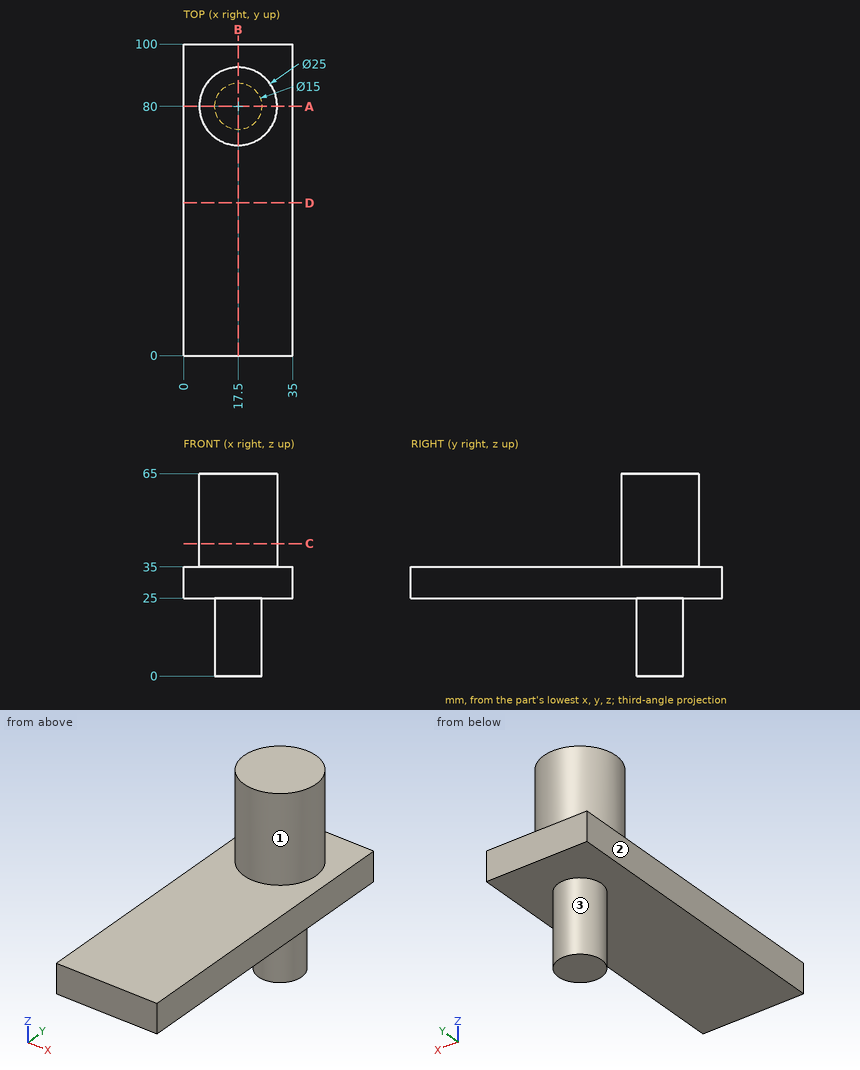
Here's the drawing with two shaded views (mm, measured from the low corner). I have some questions. A direction names the side the tool comes from. Give positions to 0.01 mm unless a question says otherwise; leave off trailing zeros. Write each loop counter-clockwise with the first axis right and the second up, starting at its lowest first coordinate (ties: lowest second). Pieces come first, ordered by that corner, then holes. Notation, with made-up numbers: (37.25, 60) - (45.25, 60) arc R13 ccw to (45.25, 80) - close; hole circle Ø7 at (31, 56). An arc over 180 degrees is marked (long way). Write item = value, one per line. Start each with the question number.
1. Imagine slicing it at A-A (y = 80). Please give me the cut outline in (x, z).
2. For pin 1 (12 mm diameter, centred on x = 21.5, z = 55, fed in from +Y); pin 2 (3 mm diameter, centred on x = 25.5, y = 15, fed in from -Z); pin 3 (1 mm diameter, centred on x = 15.5, z = 7.5, fed in from -Y), each with a flat end and sliding along its axis, tell me the tip position at first contact or that it passes through.
3. Imagine slicing it at D-D (y = 49). Please give me the cut outline in (x, z), and give its area (3 significant figures).
4. Please list where these lines run through material, in increasing order: line 1 (Z direction, x = 14.5, y = 59); line 2 (Y direction, x = 18, z = 7.5); line 3 (Y direction, x = 12.5, z = 19).
5. On a 3-axis mill with a long thin cutter (end or side, diameter ignored), from which of +Z, -Z, +X, -X, +Y, -Y can I reach the whole of each face in a straight line? I mean the marked faces 1, 2 and 3. Say none if no direction works.
6. Imagine slicing it at C-C (z = 42.5). Please give me the cut outline in (x, y).
7. Imagine slicing it at B-B (x = 17.5). Please give me the cut outline in (y, z), and give its area (4 significant figures).
Worked answers:
q1.outline = (0, 25) - (10, 25) - (10, 0) - (25, 0) - (25, 25) - (35, 25) - (35, 35) - (30, 35) - (30, 65) - (5, 65) - (5, 35) - (0, 35) - close
q2.pin_1 = 92.5
q2.pin_2 = 25
q2.pin_3 = 72.65
q3.outline = (0, 25) - (35, 25) - (35, 35) - (0, 35) - close
q3.area = 350 mm2
q4.line_1 = 25 to 35
q4.line_2 = 72.52 to 87.48
q4.line_3 = 74.41 to 85.59
q5.face_1 = +Z
q5.face_2 = +Z, -Z, -X, +Y, -Y
q5.face_3 = -Z
q6.outline = circle Ø25 at (17.5, 80)
q7.outline = (0, 25) - (72.5, 25) - (72.5, 0) - (87.5, 0) - (87.5, 25) - (100, 25) - (100, 35) - (92.5, 35) - (92.5, 65) - (67.5, 65) - (67.5, 35) - (0, 35) - close
q7.area = 2,125 mm2
